Read the model definition and answer for the solid it produces. Units are mm, in the model's axes. A direction names the side the tool comes from. Coordinates: 2 decimals unless noted, no trailing zeros. Write each loop counter-clockwise with the first axis right and the second up, starting at its lowest first coordinate (ties: lowest second). Pieces come first, ordered by that corner, then holes. Notation, with made-up numbers: (-39, -32) - (-29, -32) arc R29 ccw to (-29, -8) - close; hole circle Ø6 at (43, 56). An arc over 180 degrees is marked (long way). Use a Markdown table: item, result.
from build123d import *

# Parameters (mm, degrees)
HEX_HEAD_DEPTH                 = 45
HEAD_CHAMFER_PROFILE_OUTSIDE_W = 245.11
HEAD_CHAMFER_PROFILE_OUTSIDE_H = 229.022
HEAD_CHAMFER_PROFILE_OUTSIDE_R = 52
HEAD_TOP_CHAMFER_45DEG_DEPTH   = 45
HEAD_TOP_CHAMFER_45DEG_DRAFT   = -45
SHANK_PROFILE_50_R             = 25
SHANK_50X445_DEPTH             = 445
SHANK_END_CHAMFER_4X45DEG_SIZE = 4


with BuildPart() as part:
    # Hex Head Profile 104AF → Hex Head (new body)
    with BuildSketch(Plane(origin=(0, 0, 0), x_dir=(1, 0, 0), z_dir=(0, 1, 0))):
        Polygon((30.022213998, -52), (60.044427996, 0), (30.022213998, 52), (-30.022213998, 52), (-60.044427996, 0), (-30.022213998, -52), align=None)
    extrude(amount=HEX_HEAD_DEPTH)


with BuildPart() as head_top_chamfer_45deg_tool:
    # Head Chamfer Profile outside → Head Top Chamfer 45deg (with draft: the straight prism first)
    with BuildSketch(Plane(origin=(0, 45, 0), x_dir=(1, 0, 0), z_dir=(0, 1, 0))):
        Rectangle(HEAD_CHAMFER_PROFILE_OUTSIDE_W, HEAD_CHAMFER_PROFILE_OUTSIDE_H)
        Circle(HEAD_CHAMFER_PROFILE_OUTSIDE_R, mode=Mode.SUBTRACT)
    extrude(amount=-HEAD_TOP_CHAMFER_45DEG_DEPTH)
    # Head Top Chamfer 45deg: the draft: its side faces are tilted about the plane it starts from
    head_top_chamfer_45deg_sides = [head_top_chamfer_45deg_tool.faces().sort_by_distance(p)[0] for p in [
        (0, 22.5, 114.511),
        (122.555, 22.5, 0),
        (0, 22.5, -114.511),
        (-122.555, 22.5, 0),
        (-52, 22.5, 0),
    ]]
    draft(head_top_chamfer_45deg_sides, Plane(origin=(0, 45, 0), x_dir=(1, 0, 0), z_dir=(0, 1, 0)), HEAD_TOP_CHAMFER_45DEG_DRAFT)


with BuildPart() as part_1:
    add(part.part)

    # Head Top Chamfer 45deg: cut by head_top_chamfer_45deg_tool
    add(head_top_chamfer_45deg_tool.part, mode=Mode.SUBTRACT)

    # Shank Profile Ø50 → Shank Ø50x445 (add)
    with BuildSketch(Plane.XZ):
        with Locations(Location((0, 0, 0), (0, 0, 270))):
            Circle(SHANK_PROFILE_50_R)
    extrude(amount=SHANK_50X445_DEPTH)

    # Shank End Chamfer 4x45deg
    shank_end_chamfer_4x45deg_edges = [part_1.edges().sort_by_distance(p)[0] for p in [
        (0, -445, 25),
    ]]
    chamfer(shank_end_chamfer_4x45deg_edges, length=SHANK_END_CHAMFER_4X45DEG_SIZE)


solid = part_1.part
(1) For faces 1 (the cylindrical face through (7.509, -217.413, -23.846)), 2 (the flat face through (-44.823, 22.185, -26.364)), determine the directions among +Z, -Z, +X, -X, +Y, -Y from which every point of the face is accessible in a straight line to the end or side of a thin tool.
Report:
| item | result |
|---|---|
| face 1 | -Y |
| face 2 | -Z, -X, +Y, -Y |
(2) A cutting plane is placed at A-A, the plane y = -73. Write down the section's boundary in (x, z), and give its area (3 significant figures).
Report:
| item | result |
|---|---|
| outline | circle Ø50 at (0, 0) |
| area | 1,960 mm² |
(3) Each of these flat-tipped pins is pushed along its axis until it touches: P1, Ø4, axis at x = -18.5, y = -98.5, coming from the +Z side; P2, Ø4, axis at y = -372, z = -28, coming from the +X side; P3, Ø2, axis at y = -91.5, z = 4.5, coming from the -X side; P4, Ø6, axis at y = -385, z = 5.5, coming from the +X side. Where does it stop, or does it pass through?
Report:
| item | result |
|---|---|
| P1 | stops at z = 18.78 |
| P2 | passes through |
| P3 | stops at x = -24.75 |
| P4 | stops at x = 24.87 |
(4) Straight lines are drawn through the part: L1, parallel to Y at x = 43, z = -26.5; L2, parallel to Z at x = -2, y = -363; L3, parallel to Z at x = 17, y = -56. For each, find the intervals that lie inside material, in ascending order.
Report:
| item | result |
|---|---|
| L1 | y = 0 to 45 |
| L2 | z = -24.92 to 24.92 |
| L3 | z = -18.33 to 18.33 |
